Design review of the part shown in the three views and the two pictorial views. Dimensions are in mm from the part's minimum x, y and z. Give positions to 0.01 mm unless a question says otherwise; leave off trailing zeros. Write each loop counter-clockwise with the first axis right and the second up, starting at its lowest first coordinate (ties: lowest second). Pieces come first, ordered by that corner, then holes.
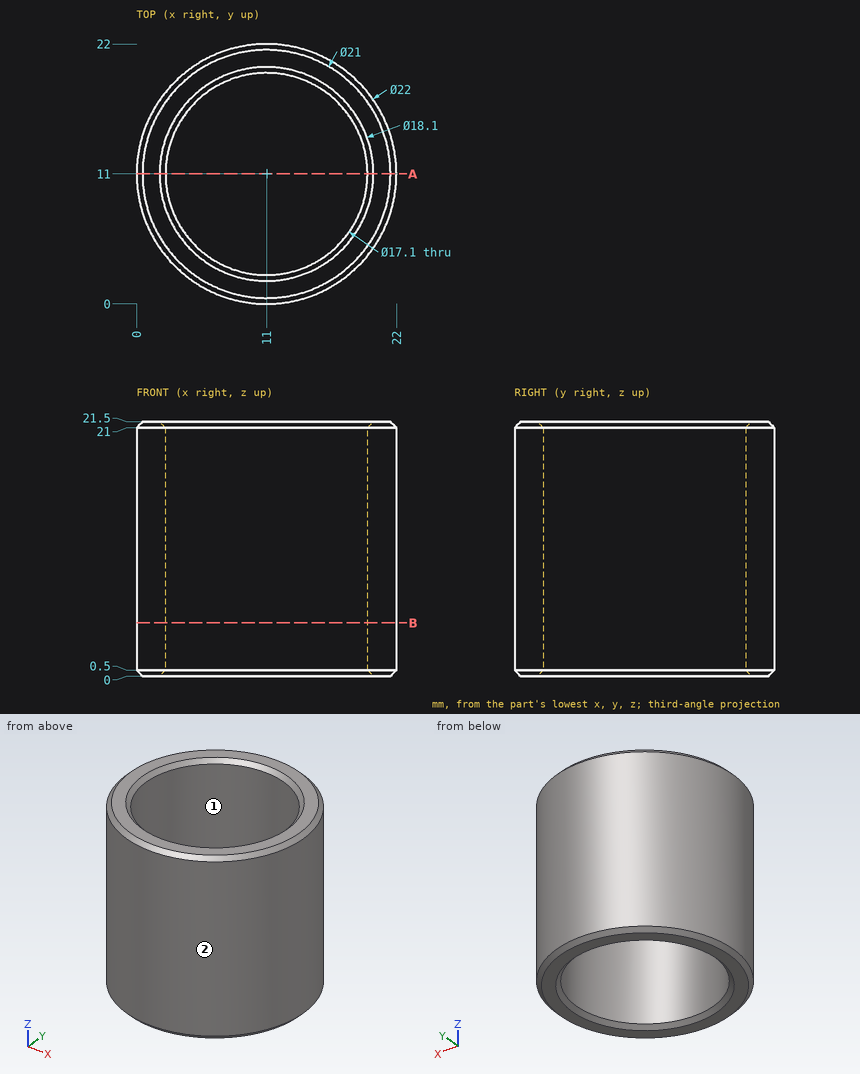
(1) Mouldability with a two-part tool opening along X and no side actions: class the marked faces 1 and 2 as pulls with the +X half, pulls with the -X half, needs draft (parallel to the pull), parting line crosses it, or undercut.
Resolved:
face 1: undercut
face 2: parting line crosses it
(2) To check wall thickness, follow L1, parallel to Y at x = 11, z = 7; L2, parallel to X at y = 15.75, z = 4.75; L3, parallel to X at y = 8.5, z = 20.5. State the ranges of each line that lie inside material, in increasing order.
Resolved:
L1: y = 0 to 2.45, 19.55 to 22
L2: x = 1.08 to 3.89, 18.11 to 20.92
L3: x = 0.29 to 2.82, 19.18 to 21.71
(3) Clearance check with flat-ended pins moving along their axes: P1, Ø1.5, axis at y = 8, z = 18.5, coming from the -X side; P2, Ø1, axis at x = 19.5, z = 17, coming from the -Y side. State where each tip first meets the part, or that it passes through.
Resolved:
P1: stops at x = 0.23
P2: stops at y = 3.45
(4) Consider section A-A, the plane y = 11. Give the boundary of the cut face in (x, z).
Resolved:
outline: (0, 0.5) - (0.5, 0) - (1.95, 0) - (2.45, 0.5) - (2.45, 21) - (1.95, 21.5) - (0.5, 21.5) - (0, 21) - close; (19.55, 0.5) - (20.05, 0) - (21.5, 0) - (22, 0.5) - (22, 21) - (21.5, 21.5) - (20.05, 21.5) - (19.55, 21) - close
(5) Consider section B-B, the plane z = 4.5. Give the boundary of the cut face in (x, y), then the cut area to 3 significant figures.
Resolved:
outline: circle Ø22 at (11, 11); hole circle Ø17.1 at (11, 11)
area: 150 mm2
